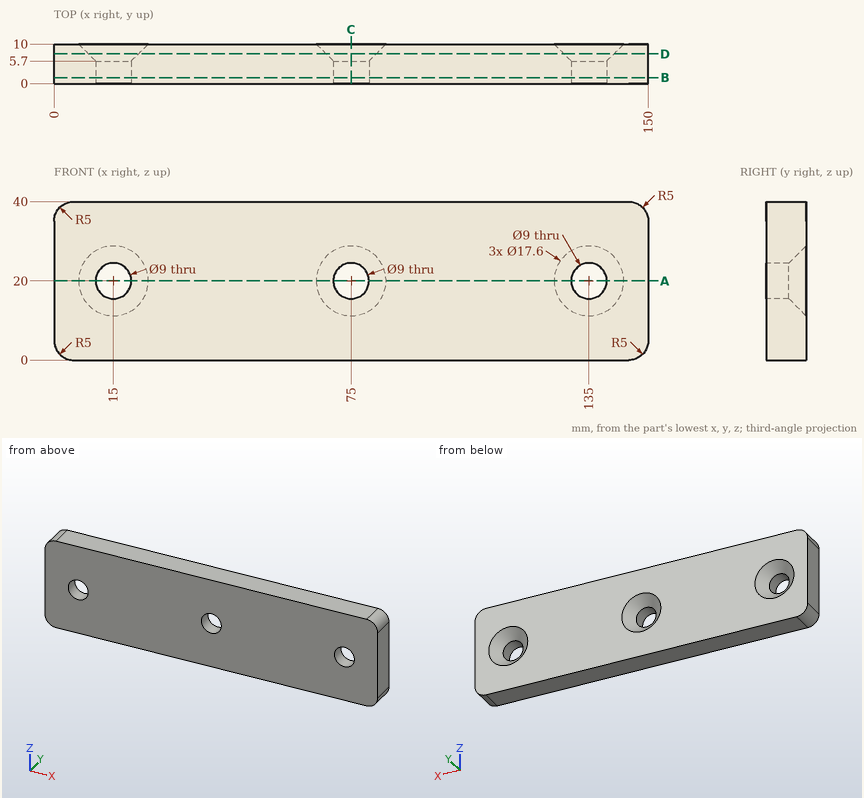
Job drawing, mm, ordinate dimensions from the low corner. One solid piece. Coordinates: 2 decimals unless noted, no trailing zeros. Write each loop counter-clockwise with the first axis right and the second up, starting at its lowest first coordinate (ties: lowest second). Pieces come first, ordered by that corner, then holes. Notation, with made-up numbers: M -11,-1.5 L 46,-1.5 A25 cw 46,18.5 Z; hole C -23,37 d1. An arc over 180 degrees is marked long. Answer as a JSON object with one key per item and string values. Group by question number.
1) Saw through at D-D (y = 7.5). Write the cut outline in (x, z).
2) Pin check, flat tips, straight feed: pin 1 Ø5.5 at (x, z) = (75, 20) entering from +Y; pin 2 Ø1 at (y, z) = (6.5, 23.5) entering from -X; pin 3 Ø14.5 at (x, z) = (15, 20) entering from +Y. Stop position of each tip, or through.
3) Saw through at A-A (z = 20). Write the cut outline in (x, y).
4) Wall check: line 1 (X direction, y = 3.55, z = 20); line 2 (Z direction, x = 75, y = 1.2); line 3 (X direction, y = 6.5, z = 21). Give the ranges that are in metal, low to high. Write a range as from..to.
5) Saw through at C-C (x = 75). Write the cut outline in (y, z), plus the area to 3 significant figures.
6) Saw through at B-B (y = 1.5). Write the cut outline in (x, z), plus the area to 3 significant figures.
Values follow:
{
 "1": {"outline": "M 0,5 A5 ccw 5,0 L 145,0 A5 ccw 150,5 L 150,35 A5 ccw 145,40 L 5,40 A5 ccw 0,35 Z; hole C 15,20 d12.6; hole C 75,20 d12.6; hole C 135,20 d12.6"},
 "2": {"pin 1": "passes through", "pin 2": "stops at x = 0", "pin 3": "stops at y = 8.45"},
 "3": {"outline": "M 0,0 L 10.5,0 L 10.5,5.7 L 6.2,10 L 0,10 Z; M 19.5,0 L 70.5,0 L 70.5,5.7 L 66.2,10 L 23.8,10 L 19.5,5.7 Z; M 79.5,0 L 130.5,0 L 130.5,5.7 L 126.2,10 L 83.8,10 L 79.5,5.7 Z; M 139.5,0 L 150,0 L 150,10 L 143.8,10 L 139.5,5.7 Z"},
 "4": {"line 1": "x = 0..10.5, 19.5..70.5, 79.5..130.5, 139.5..150", "line 2": "z = 0..15.5, 24.5..40", "line 3": "x = 0..9.8, 20.2..69.8, 80.2..129.8, 140.2..150"},
 "5": {"outline": "M 0,0 L 10,0 L 10,11.2 L 5.7,15.5 L 0,15.5 Z; M 0,24.5 L 5.7,24.5 L 10,28.8 L 10,40 L 0,40 Z", "area": "292 mm2"},
 "6": {"outline": "M 0,5 A5 ccw 5,0 L 145,0 A5 ccw 150,5 L 150,35 A5 ccw 145,40 L 5,40 A5 ccw 0,35 Z; hole C 15,20 d9; hole C 75,20 d9; hole C 135,20 d9", "area": "5,790 mm2"}
}
